from build123d import *

# Parameters (mm, degrees)
SKETCH_1_R               = 30
SKETCH_1_R_2             = 16
EXTRUDE_1_DEPTH          = 2
CUT_EXTRUDE_1_DEPTH      = 43.473521163
CUT_EXTRUDE_1_DEPTH_BACK = 43.473521163


with BuildPart() as part:
    # 草图1 → 凸台-拉伸1 (new body)
    with BuildSketch(Plane(origin=(0, 0, 0), x_dir=(1, 0, 0), z_dir=(0, 1, 0))):
        with Locations(Location((0, 0, 0), (0, 0, 270))):
            Circle(SKETCH_1_R)
        with Locations(Location((0, 0, 0), (0, 0, 270))):
            Circle(SKETCH_1_R_2, mode=Mode.SUBTRACT)
    extrude(amount=EXTRUDE_1_DEPTH)

    # 草图2 → 切除-拉伸1 (cut, two sides: drawn at the far end of the back side and taken through both)
    with BuildSketch(Plane(origin=(0, 2, 0), x_dir=(1, 0, 0), z_dir=(0, 1, 0)).offset(-CUT_EXTRUDE_1_DEPTH_BACK)):
        with BuildLine():
            ThreePointArc((6.858704695, 25.597034397), (0, 26.5), (-6.858704695, 25.597034397))
            ThreePointArc((-6.858704695, 25.597034397), (-9.333578429, 21.310427347), (-5.046971379, 18.835553613))
            ThreePointArc((-5.046971379, 18.835553613), (0, 19.5), (5.046971379, 18.835553613))
            ThreePointArc((5.046971379, 18.835553613), (9.333578429, 21.310427347), (6.858704695, 25.597034397))
        make_face()
        with BuildLine():
            ThreePointArc((25.597034397, 6.858704695), (22.9496732, 13.25), (18.738329701, 18.738329701))
            ThreePointArc((18.738329701, 18.738329701), (13.788582233, 18.738329701), (13.788582233, 13.788582233))
            ThreePointArc((13.788582233, 13.788582233), (16.887495374, 9.75), (18.835553613, 5.046971379))
            ThreePointArc((18.835553613, 5.046971379), (23.122160663, 2.572097645), (25.597034397, 6.858704695))
        make_face()
        with BuildLine():
            ThreePointArc((18.738329701, -18.738329701), (22.9496732, -13.25), (25.597034397, -6.858704695))
            ThreePointArc((25.597034397, -6.858704695), (23.122160663, -2.572097645), (18.835553613, -5.046971379))
            ThreePointArc((18.835553613, -5.046971379), (16.887495374, -9.75), (13.788582233, -13.788582233))
            ThreePointArc((13.788582233, -13.788582233), (13.788582233, -18.738329701), (18.738329701, -18.738329701))
        make_face()
        with BuildLine():
            ThreePointArc((-6.858704695, -25.597034397), (0, -26.5), (6.858704695, -25.597034397))
            ThreePointArc((6.858704695, -25.597034397), (9.333578429, -21.310427347), (5.046971379, -18.835553613))
            ThreePointArc((5.046971379, -18.835553613), (0, -19.5), (-5.046971379, -18.835553613))
            ThreePointArc((-5.046971379, -18.835553613), (-9.333578429, -21.310427347), (-6.858704695, -25.597034397))
        make_face()
        with BuildLine():
            ThreePointArc((-25.597034397, -6.858704695), (-22.9496732, -13.25), (-18.738329701, -18.738329701))
            ThreePointArc((-18.738329701, -18.738329701), (-13.788582233, -18.738329701), (-13.788582233, -13.788582233))
            ThreePointArc((-13.788582233, -13.788582233), (-16.887495374, -9.75), (-18.835553613, -5.046971379))
            ThreePointArc((-18.835553613, -5.046971379), (-23.122160663, -2.572097645), (-25.597034397, -6.858704695))
        make_face()
        with BuildLine():
            ThreePointArc((-18.738329701, 18.738329701), (-22.9496732, 13.25), (-25.597034397, 6.858704695))
            ThreePointArc((-25.597034397, 6.858704695), (-23.122160663, 2.572097645), (-18.835553613, 5.046971379))
            ThreePointArc((-18.835553613, 5.046971379), (-16.887495374, 9.75), (-13.788582233, 13.788582233))
            ThreePointArc((-13.788582233, 13.788582233), (-13.788582233, 18.738329701), (-18.738329701, 18.738329701))
        make_face()
    extrude(amount=CUT_EXTRUDE_1_DEPTH + CUT_EXTRUDE_1_DEPTH_BACK, mode=Mode.SUBTRACT)


solid = part.part
Build history of the part. All positions in model axes, mm. Round coordinates to 2 decimals unless told otherwise and drop trailing zeros. Loops run counter-clockwise (first coordinate to the right, second up) from the corner with the lowest first, then second, coordinate; pieces in that order, holes last. Notation, with made-up numbers: (77, 64.25) -> (97, 64.25) arc R29 cw to (97, 84.25) -> close; hole circle Ø5 at (1.5, -34). An arc over 180 degrees is marked (long way). One line per item, written item: value. Start each with the question number.
Q1. Cut at D-D on x = -17.5. List the corners of the cut face in (y, z).
Q2. Drop a flat-ended pin along its axis: pin 1 Ø1 at (y, z) = (0.5, -14.5) entering from +X. Give the stop position or say it passes through.
Q3. Cut at C-C on y = 1. List the corners of the cut face in (x, z), plus the area to 3 significant figures.
Q4. Cut at A-A on z = 0. List the corners of the cut face in (x, y).
Q5. Probe line 1 along X through (y, z) = (1.55, 0); line 2 along Z through (x, y) = (17, 0.45); line 3 along Z through (x, y) = (5.5, 0.9). List the from-to ranges inside material, lowest first.
Q6. Cut at B-B on x = 0. List the corners of the cut face in (y, z), plus the area to 3 significant figures.
Q7. Two-plate mould, pull along X, no slides. Class faces 1 (the face through (16, 0, 4)), 2 (the face through (-16.92, 0.99, -9.69)): released by +X, released by -X, zero draft, split by the parting line, or undercut.
Computed:
1. outline: (0, -24.37) -> (2, -24.37) -> (2, -19.54) -> (0, -19.54) -> close; (0, -8.6) -> (2, -8.6) -> (2, 8.6) -> (0, 8.6) -> close; (0, 19.54) -> (2, 19.54) -> (2, 24.37) -> (0, 24.37) -> close
2. pin 1: x = 26.53
3. outline: circle Ø60 at (0, 0); hole (-25.6, -6.86) arc R26.5 ccw to (-18.74, -18.74) arc R3.5 ccw to (-13.79, -13.79) arc R19.5 cw to (-18.84, -5.05) arc R3.5 ccw to start; hole (-25.6, 6.86) arc R3.5 ccw to (-18.84, 5.05) arc R19.5 cw to (-13.79, 13.79) arc R3.5 ccw to (-18.74, 18.74) arc R26.5 ccw to start; hole circle Ø32 at (0, 0); hole (-6.86, -25.6) arc R26.5 ccw to (6.86, -25.6) arc R3.5 ccw to (5.05, -18.84) arc R19.5 cw to (-5.05, -18.84) arc R3.5 ccw to start; hole (-6.86, 25.6) arc R3.5 ccw to (-5.05, 18.84) arc R19.5 cw to (5.05, 18.84) arc R3.5 ccw to (6.86, 25.6) arc R26.5 ccw to start; hole (13.79, -13.79) arc R3.5 ccw to (18.74, -18.74) arc R26.5 ccw to (25.6, -6.86) arc R3.5 ccw to (18.84, -5.05) arc R19.5 cw to start; hole (13.79, 13.79) arc R19.5 cw to (18.84, 5.05) arc R3.5 ccw to (25.6, 6.86) arc R26.5 ccw to (18.74, 18.74) arc R3.5 ccw to start
3. area: 1,290 mm²
4. outline: (-30, 0) -> (-16, 0) -> (-16, 2) -> (-30, 2) -> close; (16, 0) -> (30, 0) -> (30, 2) -> (16, 2) -> close
5. line 1: -30 to -16, 16 to 30
5. line 2: -24.72 to -19.69, -9.55 to 9.55, 19.69 to 24.72
5. line 3: -29.49 to -25.92, -18.75 to -15.02, 15.02 to 18.75, 25.92 to 29.49
6. outline: (0, -30) -> (2, -30) -> (2, -26.5) -> (0, -26.5) -> close; (0, -19.5) -> (2, -19.5) -> (2, -16) -> (0, -16) -> close; (0, 16) -> (2, 16) -> (2, 19.5) -> (0, 19.5) -> close; (0, 26.5) -> (2, 26.5) -> (2, 30) -> (0, 30) -> close
6. area: 28.0 mm²
7. face 1: zero draft
7. face 2: undercut
